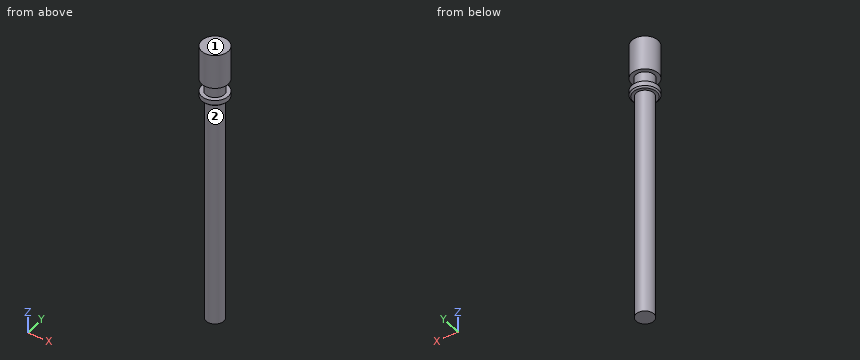
from build123d import *

# Parameters (mm, degrees)
SKETCH1_R           = 3
BOSS_EXTRUDE1_DEPTH = 96
SKETCH2_R           = 4.5
BOSS_EXTRUDE2_DEPTH = 18
CUT_EXTRUDE1_START  = -11.6
SKETCH3_OUTSIDE_W   = 30.368
SKETCH3_OUTSIDE_H   = 30.368
SKETCH3_OUTSIDE_R   = 3.15
CUT_EXTRUDE1_DEPTH  = 4.3
CHAMFER1_SIZE       = 0.5


with BuildPart() as part:
    # Sketch1 → Boss-Extrude1 (new body)
    with BuildSketch(Plane.XY):
        Circle(SKETCH1_R)
    extrude(amount=BOSS_EXTRUDE1_DEPTH)

    # Sketch2 → Boss-Extrude2 (add)
    with BuildSketch(Plane.XY.offset(96)):
        Circle(SKETCH2_R)
    extrude(amount=-BOSS_EXTRUDE2_DEPTH)

    # Sketch3 outside → Cut-Extrude1 (cut)
    with BuildSketch(Plane.XY.offset(96).offset(CUT_EXTRUDE1_START)):
        Rectangle(SKETCH3_OUTSIDE_W, SKETCH3_OUTSIDE_H)
        Circle(SKETCH3_OUTSIDE_R, mode=Mode.SUBTRACT)
    extrude(amount=-CUT_EXTRUDE1_DEPTH, mode=Mode.SUBTRACT)

    # Chamfer1
    chamfer1_edges = [part.edges().sort_by_distance(p)[0] for p in [
        (-4.5, 0, 78),
    ]]
    chamfer(chamfer1_edges, length=CHAMFER1_SIZE)


solid = part.part
Part model, mm, in its own coordinate system. Face numbers are marked on the shaded views. A direction names the side the tool comes from. Give positions to 0.01 mm unless a question says otherwise; leave off trailing zeros. Loops run counter-clockwise (first coordinate to the right, second up) from the corner with the lowest first, then second, coordinate; pieces in that order, holes last.
(1) Pin check, flat tips, straight feed: pin 1 (1.5 mm diameter, centred on x = -2.5, z = 68, fed in from +Y); pin 2 (2 mm diameter, centred on x = -1, z = 18, fed in from +Y); pin 3 (3 mm diameter, centred on x = 1, z = 48.5, fed in from -Y). Stop position of each tip, or through.
Return value:
pin 1: stops at y = 2.44
pin 2: stops at y = 3
pin 3: stops at y = -3
(2) Band-saw the part on A-A (x = 0). Write the cut outline in (y, z), and give its area (3 significant figures).
Return value:
outline: (-4.5, 78.5) - (-4, 78) - (-3, 78) - (-3, 0) - (3, 0) - (3, 78) - (4, 78) - (4.5, 78.5) - (4.5, 80.1) - (3.15, 80.1) - (3.15, 84.4) - (4.5, 84.4) - (4.5, 96) - (-4.5, 96) - (-4.5, 84.4) - (-3.15, 84.4) - (-3.15, 80.1) - (-4.5, 80.1) - close
area: 618 mm2
(3) 3-axis set-ups, long thin cutter, end or side, ignore diameter. For the marked faces 1 and 2: which of +Z, -Z, +X, -X, +Y, -Y reach the whole face in a straight line?
Return value:
face 1: +Z, +X, -X, +Y, -Y
face 2: -Z
(4) Drill centre lines: line 1 along Z through (x, y) = (2, -2.5); line 2 along X through (y, z) = (0, 53); line 3 along Y through (x, z) = (-0.25, 44.5). Where is each one in solid material? Low to high.
Return value:
line 1: z = 78 to 80.1, 84.4 to 96
line 2: x = -3 to 3
line 3: y = -2.99 to 2.99
(5) Band-saw the part on C-C (z = 48.5). Write the cut outline in (x, y), and give its area (3 significant figures).
Return value:
outline: circle Ø6 at (0, 0)
area: 28.3 mm2
(6) Band-saw the part on D-D (z = 86). Write the cut outline in (x, y).
Return value:
outline: circle Ø9 at (0, 0)
